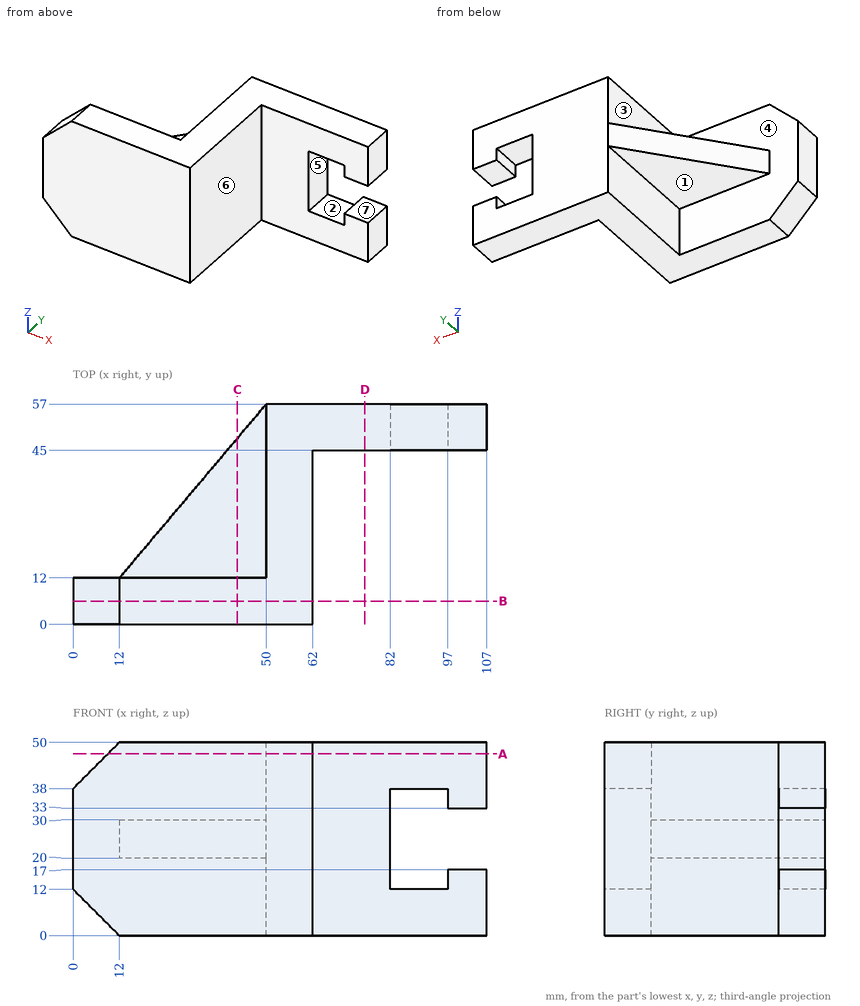
Answer from the drawing. Dimensions are ordinates in mm from the lowest x, y and z of the part. A direction names the side the tool comes from. Give positions to 0.01 mm unless a question says otherwise; leave off trailing zeros. Write each loop counter-clockwise with the first axis right and the second up, starting at its lowest first coordinate (ties: lowest second). Pieces come first, ordered by that corner, then holes.
1) Section C-C (x = 42.5) is taken. Write down the section's boundary in (y, z).
2) Given P1, Ø2, axis at y = 43, z = 26.5, coming from the -X side; P2, Ø3.5, axis at y = 49.5, z = 29, coming from the +X side; P3, Ø4, axis at y = 49, z = 35, coming from the -X side, each flat-ended and moving along its own axis, determine where each tip first touches the part or whether it passes through.
3) Section D-D (x = 75.5) is taken. Write down the section's boundary in (y, z).
4) Section A-A (z = 47) is taken. Write down the section's boundary in (x, y), and give its area (3 significant figures).
5) Find the intervals of material crossed by L1, parallel to Y at x = 76.5, z = 47.5; L2, parallel to X at y = 26.5, z = 33; L3, parallel to Y at x = 7, z = 44, in increasing order.
6) For a pull along X with two mould halves and no side action, classify the marked faces 5, 6 and 7 as pulls with the +X half, pulls with the -X half, needs draft (parallel to the pull), parting line crosses it, or undercut.
7) A tool of negligible diameter and unlimited length cuts with its end or side. For the marked faces 1, 2, 3 and 4, from which of +Z, -Z, +X, -X, +Y, -Y can it reach the whole face along a straight path? Write none if from no direction.
8) Section B-B (y = 6) is taken. Write down the section's boundary in (x, z).
Response:
1. outline: (0, 0) - (12, 0) - (12, 20) - (48.12, 20) - (48.12, 30) - (12, 30) - (12, 50) - (0, 50) - close
2. P1: stops at x = 37.33
2. P2: stops at x = 82
2. P3: stops at x = 50
3. outline: (45, 0) - (57, 0) - (57, 50) - (45, 50) - close
4. outline: (9, 0) - (62, 0) - (62, 45) - (107, 45) - (107, 57) - (50, 57) - (50, 12) - (9, 12) - close
4. area: 1,720 mm2
5. L1: y = 45 to 57
5. L2: x = 50 to 62
5. L3: y = 0 to 12
6. face 5: undercut
6. face 6: pulls with the +X half
6. face 7: needs draft
7. face 1: -Z, -X, +Y
7. face 2: +Y, -Y
7. face 3: +Z, -X, +Y
7. face 4: -X, +Y
8. outline: (0, 12) - (12, 0) - (62, 0) - (62, 50) - (12, 50) - (0, 38) - close
